```python
from build123d import *

# Parameters (mm, degrees)
HEX_NUT_PROFILE_R  = 10
HEX_NUT_BODY_DEPTH = 10


with BuildPart() as part:
    # Hex Nut Profile → Hex Nut Body (new, symmetric)
    with BuildSketch(Plane(origin=(0, 0, 0), x_dir=(1, 0, 0), z_dir=(0, 1, 0))):
        Polygon((28.867513459, 0), (14.43375673, 25), (-14.43375673, 25), (-28.867513459, 0), (-14.43375673, -25), (14.43375673, -25), align=None)
        with Locations(Location((0, 0, 0), (0, 0, 270))):
            Circle(HEX_NUT_PROFILE_R, mode=Mode.SUBTRACT)
    extrude(amount=HEX_NUT_BODY_DEPTH, both=True)


solid = part.part
```
Source: CAD feature listing. Evaluate the final solid. Frame: model axes, mm. Coordinates: 2 decimals unless noted, no trailing zeros. Loops run counter-clockwise (first coordinate to the right, second up) from the corner with the lowest first, then second, coordinate; pieces in that order, holes last. Notation, with made-up numbers: M -30,25.5 L -13,25.5 A15 ccw -13,46.5 Z; hole C 49.25,19.25 d7. An arc over 180 degrees is marked long. Use a Markdown table: item, result. Add a question column.
Q1. Section query B-B, the plane y = 3.5. Return loops of the section in (x, z).
Q2. Section query C-C, the plane z = 17. Return loops of the section in (x, y), and give its area (3 significant figures).
Q3. First-contact query: pin 1 (12 mm diameter, centred on x = 0, z = 0, fed in from +Y); pin 2 (4 mm diameter, centred on y = -3, z = -10, fed in from +X); pin 3 (12 mm diameter, centred on y = 5.5, z = -17.5, fed in from -X). Flat tips, straight axial feed; report the tip coordinate or a pass-through.
Q4. Section query D-D, the plane x = 8.5. Return loops of the section in (y, z).
Q5. Section query A-A, the plane x = 0. Return loops of the section in (y, z).
Q6. Material intervals for L1, parallel to X at y = 4.25, z = 0; L2, parallel to Z at x = -0.5, y = -6.75; L3, parallel to X at y = -4.75, z = -3, sorted ascending.
Q7. Draft query along X for faces 1 (the flat face through (12, -10, 0)), 2 (the flat face through (-21.75, 0.14, 12.33)), 3 (the cylindrical face through (-9.76, -0.14, -2.17)). Return one class per face: pulls with the +X half, pulls with the -X half, needs draft (parallel to the pull), parting line crosses it, or undercut.
Result:
| question | item | result |
|---|---|---|
| 1 | outline | M -28.87,0 L -14.43,-25 L 14.43,-25 L 28.87,0 L 14.43,25 L -14.43,25 Z; hole C 0,0 d20 |
| 2 | outline | M -19.05,-10 L 19.05,-10 L 19.05,10 L -19.05,10 Z |
| 2 | area | 762 mm2 |
| 3 | pin 1 | passes through |
| 3 | pin 2 | stops at x = 24.25 |
| 3 | pin 3 | stops at x = -22.23 |
| 4 | outline | M -10,-25 L 10,-25 L 10,-5.27 L -10,-5.27 Z; M -10,5.27 L 10,5.27 L 10,25 L -10,25 Z |
| 5 | outline | M -10,-25 L 10,-25 L 10,-10 L -10,-10 Z; M -10,10 L 10,10 L 10,25 L -10,25 Z |
| 6 | L1 | x = -28.87 to -10, 10 to 28.87 |
| 6 | L2 | z = -25 to -9.99, 9.99 to 25 |
| 6 | L3 | x = -27.14 to -9.54, 9.54 to 27.14 |
| 7 | face 1 | needs draft |
| 7 | face 2 | pulls with the -X half |
| 7 | face 3 | undercut |
